Design review of the part shown in the three views and the two pictorial views. Dimensions are in mm from the part's minimum x, y and z. A direction names the side the tool comes from. Round coordinates to 2 decimals unless told otherwise and drop trailing zeros. Order: outer loops, then holes, each group sorted by start corner. A loop starts at its lowest first (then second) coordinate and runs counter-clockwise, first axis right, second up. Notation, with made-up numbers: M 50,-14.75 L 65,-14.75 A14 ccw 65,-2.75 Z; hole C 75,48 d10. An arc over 180 degrees is marked long. Use a Markdown table: item, result. Add a question column.
(1) Machinability: for the marked faces 1 and 2, which of the approach directions +Z, -Z, +X, -X, +Y, -Y give a long, thin tool a straight path to every point of the face, cutting with its end or side? Answer none if there is none.
(2) Take a section at B-B (z = 8). Write out the cut boundary in (x, y), then the cut area to 3 significant figures.
(3) The part is to be moulded in two halves that separate along Y. For the marked faces 3, 4 and 5, say which applies: released by +Y, released by -Y, zero draft, split by the parting line, or undercut.
(4) For pin 1 (3 mm diameter, centred on x = 14, y = 6.5, fed in from +Z); pin 2 (6 mm diameter, centred on y = 9.5, z = 8.5, fed in from +X); pin 3 (2 mm diameter, centred on x = 13.5, y = 7.5, fed in from -Z), all flat-tipped, find the tip position at first contact; note any pin that passes through.
(5) Take a section at C-C (y = 6.5). Write out the cut boundary in (x, z), then the cut area to 3 significant figures.
(6) To check wall thickness, follow probe 1 along Z at (x, y) = (8, 8.5); probe 2 along Y at (x, z) = (13.5, 12.5); probe 3 along Z at (x, y) = (3.25, 6.5). State the ranges of each line that lie inside material, in increasing order. Write a range as from..to.
(7) Take a section at A-A (x = 8). Write out the cut boundary in (y, z), then the cut area to 3 significant figures.
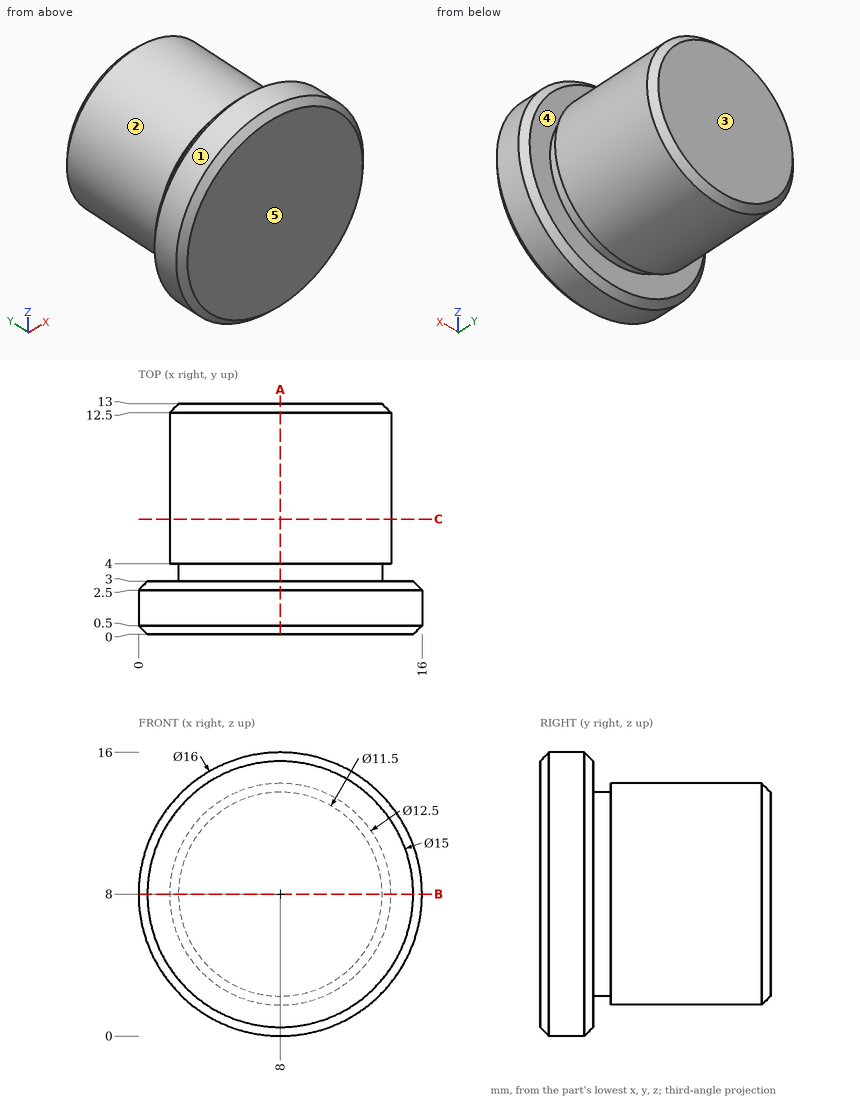
Verdict:
| question | item | result |
|---|---|---|
| 1 | face 1 | +Y, -Y |
| 1 | face 2 | +Y |
| 2 | outline | M 0,0.5 L 0.5,0 L 15.5,0 L 16,0.5 L 16,2.5 L 15.5,3 L 13.75,3 L 13.75,4 L 14.25,4 L 14.25,12.5 L 13.75,13 L 2.25,13 L 1.75,12.5 L 1.75,4 L 2.25,4 L 2.25,3 L 0.5,3 L 0,2.5 Z |
| 2 | area | 171 mm^2 |
| 3 | face 3 | released by +Y |
| 3 | face 4 | undercut |
| 3 | face 5 | released by -Y |
| 4 | pin 1 | stops at z = 12.34 |
| 4 | pin 2 | stops at x = 14.25 |
| 4 | pin 3 | stops at z = 3.66 |
| 5 | outline | C 8,8 d12.5 |
| 5 | area | 123 mm^2 |
| 6 | probe 1 | z = 1.75..14.25 |
| 6 | probe 2 | y = 0..3 |
| 6 | probe 3 | z = 3.94..12.06 |
| 7 | outline | M 0,0.5 L 0.5,0 L 2.5,0 L 3,0.5 L 3,2.25 L 4,2.25 L 4,1.75 L 12.5,1.75 L 13,2.25 L 13,13.75 L 12.5,14.25 L 4,14.25 L 4,13.75 L 3,13.75 L 3,15.5 L 2.5,16 L 0.5,16 L 0,15.5 Z |
| 7 | area | 171 mm^2 |
